For this review, take the finished solid that the model builds, in its own axes (mm). A direction names the side the tool comes from. Coordinates: 2 decimals unless noted, no trailing zeros. Write each loop counter-clockwise with the first axis right and the second up, starting at its lowest first coordinate (ties: lowest second). Pieces come first, ordered by that corner, then holes. Notation, with made-up numbers: (10.25, 26.5) - (23.25, 26.5) arc R24 cw to (23.25, 55.5) - close; hole circle Ø10 at (-1.5, -25). An arc over 180 degrees is marked (long way). Write each question's results on one line, items separated by ' | '.
from build123d import *

# Parameters (mm, degrees)
SKETCH1_W           = 91
SKETCH1_H           = 30
BOSS_EXTRUDE1_DEPTH = 10
SKETCH2_W           = 20
SKETCH2_H           = 30
BOSS_EXTRUDE2_DEPTH = 30
CUT_EXTRUDE1_DEPTH  = 30
SKETCH5_R           = 6
CUT_EXTRUDE2_DEPTH  = 30


with BuildPart() as part:
    # Sketch1 → Boss-Extrude1 (new body)
    with BuildSketch(Plane.XY):
        Rectangle(SKETCH1_W, SKETCH1_H)
    extrude(amount=BOSS_EXTRUDE1_DEPTH)

    # Sketch2 → Boss-Extrude2 (add)
    with BuildSketch(Plane.XY.offset(10)):
        Rectangle(SKETCH2_W, SKETCH2_H)
    extrude(amount=BOSS_EXTRUDE2_DEPTH)

    # Sketch4 → Cut-Extrude1 (cut)
    with BuildSketch(Plane.ZY.offset(10)):
        with BuildLine():
            Line((27.1, 7), (22.9, 7))
            Line((22.9, 7), (22.9, 4.81170448))
            ThreePointArc((22.9, 4.81170448), (25, -5.25), (27.1, 4.81170448))
            Line((27.1, 4.81170448), (27.1, 7))
        make_face()
    extrude(amount=-CUT_EXTRUDE1_DEPTH, mode=Mode.SUBTRACT)

    # Sketch5 → Cut-Extrude2 (cut)
    with BuildSketch(Plane.XY.offset(10)):
        with Locations((-30.5, 0)):
            Circle(SKETCH5_R)
        with Locations(Location((30.5, 0, 0), (0, 0, 180))):
            Circle(SKETCH5_R)
    extrude(amount=-CUT_EXTRUDE2_DEPTH, mode=Mode.SUBTRACT)


solid = part.part
Q1. For pin 1 (3 mm diameter, centred on y = 0.5, z = 35.5, fed in from +X); pin 2 (13.5 mm diameter, centred on y = 0, z = 25, fed in from -X); pin 3 (5 mm diameter, centred on x = 17, y = -2.5, fed in from +Z), all flat-tipped, find the tip position at first contact; note any pin that passes through.
Results found:
pin 1: x = 10 | pin 2: x = -10 | pin 3: z = 10
Q2. Take a section at D-D on z = 3.5. State the section outline as (x, y) points.
Results found:
outline: (-45.5, -15) - (45.5, -15) - (45.5, 15) - (-45.5, 15) - close; hole circle Ø12 at (-30.5, 0); hole circle Ø12 at (30.5, 0)
Q3. Take a section at A-A on z = 25. State the section outline as (x, y) points.
Results found:
outline: (-10, -15) - (10, -15) - (10, -5.25) - (-10, -5.25) - close; (-10, 7) - (10, 7) - (10, 15) - (-10, 15) - close
Q4. Wall thickness on line 1 along Y through (x, z) = (30.5, 4); line 2 along Y through (x, z) = (6.25, 25); line 3 along Z through (x, y) = (0.5, 0): over which ranges is each line inside the solid? List them lowest first. Write a range as from..to.
Results found:
line 1: -15..-6, 6..15 | line 2: -15..-5.25, 7..15 | line 3: 0..19.75, 30.25..40
Q5. For faces 1 (the face through (-1, -15, 11)), 2 (the face through (0, 6, 22.9)), 3 (the face through (-10, -7, 25)), 4 (the face through (24, 0, 10)), list the 3-axis set-ups (+Z, -Z, +X, -X, +Y, -Y) from which the entire face can be reached by the end or side of a thin tool; tool diameter is ignored.
Results found:
face 1: +Z, -Z, +X, -X, -Y | face 2: +X, -X | face 3: +Z, -X, +Y, -Y | face 4: +Z, +X, +Y, -Y
Q6. Take a section at B-B on x = -30.5. State the section outline as (y, z) points.
Results found:
outline: (-15, 0) - (-6, 0) - (-6, 10) - (-15, 10) - close; (6, 0) - (15, 0) - (15, 10) - (6, 10) - close
Q7. Mouldability with a two-part tool opening along Z and no side actions: class faces 5 (the face through (10, -7, 25)), 6 (the face through (0, 6, 27.1)), 7 (the face through (0, 0, 40)), 8 (the face through (-1, 0, 0)) as pulls with the +Z half, pulls with the -Z half, needs draft (parallel to the pull), parting line crosses it, or undercut.
Results found:
face 5: needs draft | face 6: undercut | face 7: pulls with the +Z half | face 8: pulls with the -Z half
Q8. Take a section at C-C on y = 13.25. State the section outline as (x, z) points, plus the area to 3 significant figures.
Results found:
outline: (-45.5, 0) - (45.5, 0) - (45.5, 10) - (10, 10) - (10, 40) - (-10, 40) - (-10, 10) - (-45.5, 10) - close | area: 1,510 mm2
